Verification items for the finished model (mm, model axes). A direction names the side the tool comes from. Coordinates: 2 decimals unless noted, no trailing zeros. Order: outer loops, then holes, each group sorted by start corner. A loop starts at its lowest first (then second) coordinate and runs counter-clockwise, first axis right, second up.
Q1. Depth check by flat-ended pin: P1, Ø5.5, axis at x = 147.5, y = 74, coming from the -Z side; P2, Ø8, axis at y = 47, z = 105, coming from the +X side; P3, Ø9, axis at x = 428, z = 145, coming from the -Y side; P4, Ø5.5, axis at x = 146.5, y = 67, coming from the +Z side. Enter the tip coordinate at first touch or a pass-through.
Q2. Draft check along X on faces 3 (the flat face through (150, 57, 117)), 4 (the flat face through (345, 0, 113)), 5 (the flat face through (145, 57, 117)). Enter one of: pulls with the +X half, pulls with the -X half, needs draft (parallel to the pull), parting line crosses it, or undercut.
Q3. Thickness scan on line 1 (Z direction, x = 85, y = 6); line 2 (X direction, y = 87.5, z = 122); line 3 (Z direction, x = 40, y = 5). Record the ranges inside material, lowest first.
Q4. Set-up check for faces 1 (the flat face through (555, 57, 117)), 2 (the flat face through (295, 70, 117)): record each of +Z, -Z, +X, -X, +Y, -Y from which the full face is reachable in a straight line by a thin tool's end or side.
Q5. Cross-section at C-C, the plane x = 590. Record the boundary of the cut face in (y, z).
Q6. Cross-section at A-A, the plane y = 77. Record the boundary of the cut face in (x, z).
Q7. Cross-section at B-B, the plane z = 135. Record the boundary of the cut face in (x, y), and give its area (3 significant figures).
from build123d import *

# Parameters (mm, degrees)
SKETCH1_W             = 700
SKETCH1_H             = 230
BOSS_EXTRUDE1_DEPTH   = 10
M8_TAPPED_HOLE1_D     = 6.8
SKETCH8_W             = 5
SKETCH8_H             = 220
BOSS_EXTRUDE2_DEPTH   = 121
SKETCH9_W             = 5
SKETCH9_H             = 220
BOSS_EXTRUDE3_DEPTH   = 95
M8_TAPPED_HOLE3_D     = 6.8
M8_TAPPED_HOLE3_DEPTH = 19.75
M8_TAPPED_HOLE3_TIP   = 2.042926105


with BuildPart() as part:
    # Sketch1 → Boss-Extrude1 (new body)
    with BuildSketch(Plane(origin=(0, 0, 0), x_dir=(1, 0, 0), z_dir=(0, 1, 0))):
        with Locations((350, -115)):
            Rectangle(SKETCH1_W, SKETCH1_H)
    extrude(amount=BOSS_EXTRUDE1_DEPTH)

    # M8 Tapped Hole1 (through all)
    with Locations(Plane(origin=(0, 10, 0), x_dir=(1, 0, 0), z_dir=(0, 1, 0))):
        with Locations((272, -85), (272, -145), (132, -145), (132, -85), (568, -85), (568, -145), (428, -145), (428, -85)):
            Hole(M8_TAPPED_HOLE1_D / 2)

    # Sketch8 → Boss-Extrude2 (add)
    with BuildSketch(Plane(origin=(0, 10, 0), x_dir=(1, 0, 0), z_dir=(0, 1, 0))):
        with Locations((292.5, -115)):
            Rectangle(SKETCH8_W, SKETCH8_H)
        with Locations((407.5, -115)):
            Rectangle(SKETCH8_W, SKETCH8_H)
    extrude(amount=BOSS_EXTRUDE2_DEPTH)

    # Sketch9 → Boss-Extrude3 (add)
    with BuildSketch(Plane(origin=(0, 10, 0), x_dir=(1, 0, 0), z_dir=(0, 1, 0))):
        with Locations((147.5, -115)):
            Rectangle(SKETCH9_W, SKETCH9_H)
        with Locations((552.5, -115)):
            Rectangle(SKETCH9_W, SKETCH9_H)
    extrude(amount=BOSS_EXTRUDE3_DEPTH)

    # M8 Tapped Hole3
    with Locations(Plane(origin=(0, 0, 0), x_dir=(-1, 0, 0), z_dir=(0, -1, 0))):
        with Locations((-85, -35), (-40, -45), (-40, -185), (-85, -195), (-40, -115), (-85, -115)):
            Hole(M8_TAPPED_HOLE3_D / 2, depth=M8_TAPPED_HOLE3_DEPTH)
            with Locations((0, 0, -(M8_TAPPED_HOLE3_DEPTH + M8_TAPPED_HOLE3_TIP / 2))):  # 118° drill point
                Cone(0, M8_TAPPED_HOLE3_D / 2, M8_TAPPED_HOLE3_TIP, mode=Mode.SUBTRACT)


solid = part.part
Check values:
1. P1: stops at z = 5
1. P2: stops at x = 555
1. P3: stops at y = 0
1. P4: stops at z = 225
2. face 3: undercut
2. face 4: needs draft
2. face 5: pulls with the -X half
3. line 1: z = 0 to 31.6, 38.4 to 111.6, 118.4 to 191.6, 198.4 to 230
3. line 2: x = 145 to 150, 290 to 295, 405 to 410, 550 to 555
3. line 3: z = 0 to 41.6, 48.4 to 111.6, 118.4 to 181.6, 188.4 to 230
4. face 1: +Z, -Z, +X, +Y
4. face 2: +Z, -Z, +Y
5. outline: (0, 0) - (10, 0) - (10, 230) - (0, 230) - close
6. outline: (145, 5) - (150, 5) - (150, 225) - (145, 225) - close; (290, 5) - (295, 5) - (295, 225) - (290, 225) - close; (405, 5) - (410, 5) - (410, 225) - (405, 225) - close; (550, 5) - (555, 5) - (555, 225) - (550, 225) - close
7. outline: (0, 0) - (700, 0) - (700, 10) - (555, 10) - (555, 105) - (550, 105) - (550, 10) - (410, 10) - (410, 131) - (405, 131) - (405, 10) - (295, 10) - (295, 131) - (290, 131) - (290, 10) - (150, 10) - (150, 105) - (145, 105) - (145, 10) - (0, 10) - close
7. area: 9,160 mm2
